from build123d import *

# Parameters (mm, degrees)
SKETCH1_R           = 50
BOSS_EXTRUDE1_DEPTH = 100


with BuildPart() as part:
    # Sketch1 → Boss-Extrude1 (new body)
    with BuildSketch(Plane.XY):
        with BuildLine():
            Line((0, 150), (1500, 150))
            Line((1500, 150), (1500, -150))
            Line((1500, -150), (0, -150))
            ThreePointArc((0, -150), (-150, 0), (0, 150))
        make_face()
        with Locations((1000, 0)):
            Circle(SKETCH1_R, mode=Mode.SUBTRACT)
        Circle(SKETCH1_R, mode=Mode.SUBTRACT)
    extrude(amount=BOSS_EXTRUDE1_DEPTH)


solid = part.part
Could you check a few things on this model? Use its own coordinates, in mm. Give positions to 0.01 mm unless a question says otherwise; leave off trailing zeros. Write each loop counter-clockwise with the first axis right and the second up, starting at its lowest first coordinate (ties: lowest second). Pieces come first, ordered by that corner, then holes. Notation, with made-up numbers: (1, -20.5) - (21, -20.5) arc R6 cw to (21, -15.5) - close; hole circle Ø5 at (-26.5, 1.25). An arc over 180 degrees is marked (long way). Use CSV: the item, a comma, the result in double quotes. Start each with the question number.
Item 1: I want a section at C-C, the plane z = 80. Please give me the cut outline in (x, y).
Item 2: I'm going to push a flat-ended pin straight in: pin 1 (5 mm diameter, centred on x = 486.5, y = -34.5, fed in from -Z). Where does the tip first touch, or does it pass through?
Item 3: If I drill on line 1 along X through (y, z) = (5.5, 11); line 2 along X through (y, z) = (1.5, 85.5); line 3 along Y through (x, z) = (1000, 60), over which ranges is the centre line in solid material (lowest first)?
Item 4: If we mould it in two halves opening along Y, with no side actions, what happens to faces 1 (the face through (-149.964, -3.298, 49.3)), 2 (the face through (687, 2, 100)), 3 (the face through (1047.69, 15.02, 49.3))? For each: pulls with the +Y half, pulls with the -Y half, needs draft (parallel to the pull), parting line crosses it, or undercut.
Item 5: I want a section at A-A, the plane y = 0. Please give me the cut outline in (x, z).
Item 6: I want a section at B-B, the plane x = 1000. Please give me the cut outline in (y, z), then the cut area to 3 significant figures.
Findings:
1,outline,"(0, -150) - (1500, -150) - (1500, 150) - (0, 150) arc R150 ccw to start; hole circle Ø100 at (0, 0); hole circle Ø100 at (1000, 0)"
2,pin 1,"stops at z = 0"
3,line 1,"x = -149.9 to -49.7, 49.7 to 950.3, 1049.7 to 1500"
3,line 2,"x = -149.99 to -49.98, 49.98 to 950.02, 1049.98 to 1500"
3,line 3,"y = -150 to -50, 50 to 150"
4,face 1,"parting line crosses it"
4,face 2,"needs draft"
4,face 3,"undercut"
5,outline,"(-150, 0) - (-50, 0) - (-50, 100) - (-150, 100) - close; (50, 0) - (950, 0) - (950, 100) - (50, 100) - close; (1050, 0) - (1500, 0) - (1500, 100) - (1050, 100) - close"
6,outline,"(-150, 0) - (-50, 0) - (-50, 100) - (-150, 100) - close; (50, 0) - (150, 0) - (150, 100) - (50, 100) - close"
6,area,"20,000 mm2"
